Input: part model. Units: mm. Frame: model coordinates. A direction names the side the tool comes from. Give positions to 0.01 mm unless a question says otherwise; leave off trailing zeros. Write each loop counter-clockwise with the first axis right and the second up, starting at its lowest first coordinate (ties: lowest second). Pieces come first, ordered by that corner, then holes. Notation, with made-up numbers: (-16.5, 77.5) -> (3.5, 77.5) arc R21 cw to (3.5, 88.5) -> close; hole circle Ø6 at (11, 1.5). An arc over 180 degrees is marked (long way). Return JSON: item names as keys, results as strings. Group by question number.
Item 1: Set-up query: faces 5 (the face through (38, 20, 0)), 6 (the face through (38, 25, 0)). Return all of +Z, -Z, +X, -X, +Y, -Y with unobstructed straight access to the full face (end or side cutting, diameter ignored); none if empty.
Item 2: Section A-A, the plane z = 9.5. Return loops of the section in (x, y).
Item 3: Pin query (flat end, axial travel): P1, Ø2, axis at y = -18, z = 14.5, coming from the -X side. Return the tip coordinate at first contact, or that it passes through.
Item 4: Mould query, pull axis Z, two halves, no side actions, for faces 1 (the face through (37.774, 22.719, 22.594)), 2 (the face through (38, 0, -25)), 3 (the face through (38, 0, 20)), 4 (the face through (38, -25, 0)). Classes: released by +Z, released by -Z, zero draft, split by the parting line, or undercut.
Item 5: Section C-C, the plane x = 126.5. Return loops of the section in (y, z).
Item 6: Line query: line 1 (Z direction, x = -4, y = -13.5); line 2 (Z direction, x = -40, y = 18). Output: solid intervals per line, ascending. Write a range as [from, to].
from build123d import *

# Parameters (mm, degrees)
COLD_FORMED_SQUARE_HOLLOW_SECTION_GB_T_6_DEPTH = 256


with BuildPart() as part:
    # Sketch1 → Cold-formed square hollow section GB/T 6728-2002 50 X 50 X 4(1) (new body)
    with BuildSketch(Plane.YZ.offset(-88.434077868)):
        with BuildLine():
            Line((-17, -25), (17, -25))
            ThreePointArc((17, -25), (22.656854249, -22.656854249), (25, -17))
            Line((25, -17), (25, 17))
            ThreePointArc((25, 17), (22.656854249, 22.656854249), (17, 25))
            Line((17, 25), (-17, 25))
            ThreePointArc((-17, 25), (-22.656854249, 22.656854249), (-25, 17))
            Line((-25, 17), (-25, -17))
            ThreePointArc((-25, -17), (-22.656854249, -22.656854249), (-17, -25))
        make_face()
        with BuildLine():
            Line((-17, -20), (17, -20))
            ThreePointArc((17, -20), (19.121320344, -19.121320344), (20, -17))
            Line((20, -17), (20, 17))
            ThreePointArc((20, 17), (19.121320344, 19.121320344), (17, 20))
            Line((17, 20), (-17, 20))
            ThreePointArc((-17, 20), (-19.121320344, 19.121320344), (-20, 17))
            Line((-20, 17), (-20, -17))
            ThreePointArc((-20, -17), (-19.121320344, -19.121320344), (-17, -20))
        make_face(mode=Mode.SUBTRACT)
    extrude(amount=COLD_FORMED_SQUARE_HOLLOW_SECTION_GB_T_6_DEPTH)


solid = part.part
Answer below:
{
 "1": {"face 5": "+X, -X", "face 6": "+Z, -Z, +X, -X, +Y"},
 "2": {"outline": "(-88.43, -25) -> (167.57, -25) -> (167.57, -20) -> (-88.43, -20) -> close; (-88.43, 20) -> (167.57, 20) -> (167.57, 25) -> (-88.43, 25) -> close"},
 "3": {"P1": "passes through"},
 "4": {"face 1": "released by +Z", "face 2": "released by -Z", "face 3": "undercut", "face 4": "zero draft"},
 "5": {"outline": "(-25, -17) arc R8 ccw to (-17, -25) -> (17, -25) arc R8 ccw to (25, -17) -> (25, 17) arc R8 ccw to (17, 25) -> (-17, 25) arc R8 ccw to (-25, 17) -> close; hole (-20, -17) arc R3 ccw to (-17, -20) -> (17, -20) arc R3 ccw to (20, -17) -> (20, 17) arc R3 ccw to (17, 20) -> (-17, 20) arc R3 ccw to (-20, 17) -> close"},
 "6": {"line 1": "z = [-25, -20], [20, 25]", "line 2": "z = [-24.94, -19.83], [19.83, 24.94]"}
}
